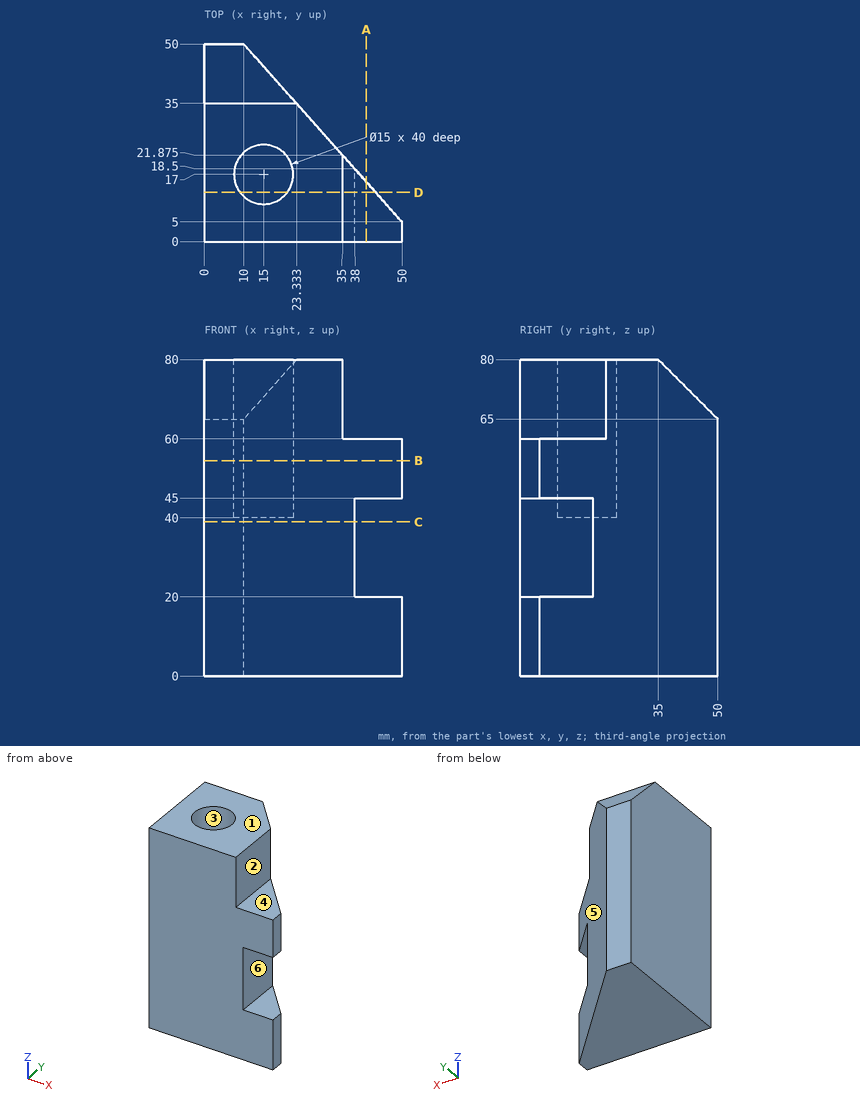
Verification items for this drawing (mm, ordinates from the low corner). A direction names the side the tool comes from. Give positions to 0.01 mm unless a question says otherwise; leave off trailing zeros. Loops run counter-clockwise (first coordinate to the right, second up) from the corner with the lowest first, then second, coordinate; pieces in that order, holes last. Notation, with made-up numbers: M -1.75,63.25 L 44.25,63.25 A24 ccw 44.25,92.25 Z; hole C 72,-15.75 d1. An arc over 180 degrees is marked long. Answer in a Markdown table with one row per item.
1) Cross-section at C-C (z = 39). Enter the section's corners in (x, y).
Solutions:
| item | result |
|---|---|
| outline | M 0,0 L 38,0 L 38,18.5 L 10,50 L 0,50 Z |
2) Mould release check, pull along X, two halves, no side actions. Record for the marked faces 1, 2 and 3: released by +X, released by -X, zero draft, split by the parting line, or undercut.
Solutions:
| item | result |
|---|---|
| face 1 | zero draft |
| face 2 | released by +X |
| face 3 | undercut |
3) Thickness scan on line 1 (X direction, y = 5.5, z = 62); line 2 (Y direction, x = 15, z = 49) (1 decimal); line 3 (Y direction, x = 9.5, z = 69). Record the ranges inside material, lowest first.
Solutions:
| item | result |
|---|---|
| line 1 | x = 0 to 35 |
| line 2 | y = 0 to 9.5, 24.5 to 44.4 |
| line 3 | y = 0 to 11.9, 22.1 to 46 |
4) Cross-section at A-A (x = 41). Enter the section's corners in (y, z) (1 decimal).
Solutions:
| item | result |
|---|---|
| outline | M 0,0 L 15.1,0 L 15.1,20 L 0,20 Z; M 0,45 L 15.1,45 L 15.1,60 L 0,60 Z |
5) Depth check by flat-ended pin: pin 1 (12 mm diameter, centred on y = 20, z = 15, fed in from +X); pin 2 (9.5 mm diameter, centred on y = 9, z = 31, fed in from +X); pin 3 (8 mm diameter, centred on x = 22, z = 25.5, fed in from +Y). Enter the tip coordinate at first touch or a pass-through.
Solutions:
| item | result |
|---|---|
| pin 1 | stops at x = 42 |
| pin 2 | stops at x = 38 |
| pin 3 | stops at y = 41 |
6) Cross-section at D-D (y = 12.5). Enter the section's corners in (x, z).
Solutions:
| item | result |
|---|---|
| outline | M 0,0 L 43.33,0 L 43.33,20 L 38,20 L 38,45 L 43.33,45 L 43.33,60 L 35,60 L 35,80 L 21,80 L 21,40 L 9,40 L 9,80 L 0,80 Z |
7) Cross-section at B-B (z = 54.5). Enter the section's corners in (x, y).
Solutions:
| item | result |
|---|---|
| outline | M 0,0 L 50,0 L 50,5 L 10,50 L 0,50 Z; hole C 15,17 d15 |
8) Tool access check on the marked faces 4, 5 and 6. Record the directions out of +Z, -Z, +X, -X, +Y, -Y that give a thin tool (end or side, any length) a straight path to the whole face; none if there is none.
Solutions:
| item | result |
|---|---|
| face 4 | +Z, +X, +Y, -Y |
| face 5 | +Z, -Z, +X, +Y |
| face 6 | +X, +Y, -Y |
